Read the model definition and answer for the solid it produces. Units are mm, in the model's axes. A direction names the side the tool comes from. Coordinates: 2 decimals unless noted, no trailing zeros. Write each loop counter-clockwise with the first axis right and the second up, starting at its lowest first coordinate (ties: lowest second). Pieces come first, ordered by that corner, then holes.
1) The part is cut by section C-C (x = -21). Determine the outline of the cut face in (y, z), then the cut area to 3 significant figures.
2) Determine the mould class of faces 6 (the face through (-20.6, 18.5, 3.5)), 7 (the face through (-16, 10, 10)), 8 (the face through (-25, 10, 5)) for opening direction X: +X half, -X half, draft (parallel to the pull), parting line (faces both ways), or undercut.
3) The part is cut by section A-A (y = 16). Determine the outline of the cut face in (x, z).
4) The part is cut by section B-B (z = 6). Determine the outline of the cut face in (x, y).
5) Each of these flat-tipped pins is pushed along its axis until it touches: pin 1 Ø2.5 at (x, y) = (19.5, 16.5) entering from -Z; pin 2 Ø5.5 at (x, z) = (21, 8) entering from +Y; pin 3 Ø1.5 at (x, y) = (-4, 13.5) entering from +Z; pin 4 Ø2.5 at (x, y) = (-19.5, 7.5) entering from -Z. Where does it stop, or does it pass through?
6) Which of the six approach directions +Z, -Z, +X, -X, +Y, -Y give full straight-line access (tool end or side, diameter ignored) to faces 1 (the face through (20, 17, 3)), 2 (the face through (21, 15, 5)), 3 (the face through (-22.19, 12.88, 13.33)), 4 (the face through (16.305, 5.968, -6.563)), 5 (the face through (16, 9, 10))?
7) The part is cut by section D-D (y = 1.75). Determine the outline of the cut face in (x, z).
8) Find the intervals of material crossed by line 1 (Y direction, x = 20, z = -7); line 2 (Y direction, x = -21, z = 13.2); line 3 (X direction, y = 8.25, z = -1), in increasing order.
from build123d import *

# Parameters (mm, degrees)
BOSS_EXTRUDE1_DEPTH   = 15
CHAMFER1_SIZE         = 10
CHAMFER1_SIZE2        = 15
CHAMFER2_SIZE         = 15
CHAMFER2_SIZE2        = 10
SKETCH2_R             = 2.25
CUT_EXTRUDE1_DEPTH    = 36
SKETCH3_R             = 4
CUT_EXTRUDE2_DEPTH    = 13
SKETCH12_R            = 3
CUT_EXTRUDE7_DEPTH    = 4.2
M3_TAPPED_HOLE1_D     = 2.5
M3_TAPPED_HOLE1_DEPTH = 7.5
M3_TAPPED_HOLE1_TIP   = 0.751075774
M3_TAPPED_HOLE2_D     = 2.5
M3_TAPPED_HOLE2_DEPTH = 7.5
M3_TAPPED_HOLE2_TIP   = 0.751075774
BOSS_EXTRUDE3_START   = 4
SKETCH17_W            = 9
SKETCH17_H            = 13
SKETCH17_R            = 3
BOSS_EXTRUDE3_DEPTH   = 4
SKETCH18_R            = 5
CUT_EXTRUDE8_DEPTH    = 8.2
CHAMFER3_SIZE         = 1


with BuildPart() as part:
    # Sketch1 → Boss-Extrude1 (new body)
    with BuildSketch(Plane(origin=(0, 0, 0), x_dir=(1, 0, 0), z_dir=(0, 1, 0))):
        Polygon((-25, 16), (25, 16), (25, -16), (16, -16), (16, -3), (-16, -3), (-16, -16), (-25, -16), align=None)
    extrude(amount=BOSS_EXTRUDE1_DEPTH)

    # Chamfer1
    chamfer1_edges = [part.edges().sort_by_distance(p)[0] for p in [
        (25, 7.5, -16),
    ]]
    chamfer1_side = [part.faces().sort_by_distance(p)[0] for p in [
        (25, 7.5, 0),
    ]]
    chamfer(chamfer1_edges, length=CHAMFER1_SIZE, length2=CHAMFER1_SIZE2, reference=chamfer1_side[0])

    # Chamfer2
    chamfer2_edges = [part.edges().sort_by_distance(p)[0] for p in [
        (-25, 7.5, -16),
    ]]
    chamfer2_side = [part.faces().sort_by_distance(p)[0] for p in [
        (-7.5, 7.5, -16),
    ]]
    chamfer(chamfer2_edges, length=CHAMFER2_SIZE, length2=CHAMFER2_SIZE2, reference=chamfer2_side[0])

    # Sketch2 → Cut-Extrude1 (cut)
    with BuildSketch(Plane(origin=(0, 0, -16), x_dir=(-1, 0, 0), z_dir=(0, 0, -1))):
        with Locations((-20, 7.5)):
            Circle(SKETCH2_R)
        with Locations((20, 7.5)):
            Circle(SKETCH2_R)
    extrude(amount=-CUT_EXTRUDE1_DEPTH, mode=Mode.SUBTRACT)

    # Sketch3 → Cut-Extrude2 (cut)
    with BuildSketch(Plane(origin=(0, 0, -16), x_dir=(-1, 0, 0), z_dir=(0, 0, -1))):
        with Locations((-20, 7.5)):
            Circle(SKETCH3_R)
        with Locations((20, 7.5)):
            Circle(SKETCH3_R)
    extrude(amount=-CUT_EXTRUDE2_DEPTH, mode=Mode.SUBTRACT)

    # Sketch12 → Cut-Extrude7 (cut)
    with BuildSketch(Plane(origin=(0, 15, 0), x_dir=(1, 0, 0), z_dir=(0, 1, 0))):
        with Locations(Location((-21, -8, 0), (0, 0, 270))):
            Circle(SKETCH12_R)
        with Locations(Location((21, -8, 0), (0, 0, 270))):
            Circle(SKETCH12_R)
    extrude(amount=-CUT_EXTRUDE7_DEPTH, mode=Mode.SUBTRACT)

    # M3 Tapped Hole1
    with Locations(Plane(origin=(-21, 12.5, 16), x_dir=(1, 0, 0), z_dir=(0, 0, 1))):
        with Locations((0, 0)):
            Hole(M3_TAPPED_HOLE1_D / 2, depth=M3_TAPPED_HOLE1_DEPTH)
            with Locations((0, 0, -(M3_TAPPED_HOLE1_DEPTH + M3_TAPPED_HOLE1_TIP / 2))):  # 118° drill point
                Cone(0, M3_TAPPED_HOLE1_D / 2, M3_TAPPED_HOLE1_TIP, mode=Mode.SUBTRACT)

    # M3 Tapped Hole2
    with Locations(Plane(origin=(21, 12.5, 16), x_dir=(1, 0, 0), z_dir=(0, 0, 1))):
        with Locations((0, 0)):
            Hole(M3_TAPPED_HOLE2_D / 2, depth=M3_TAPPED_HOLE2_DEPTH)
            with Locations((0, 0, -(M3_TAPPED_HOLE2_DEPTH + M3_TAPPED_HOLE2_TIP / 2))):  # 118° drill point
                Cone(0, M3_TAPPED_HOLE2_D / 2, M3_TAPPED_HOLE2_TIP, mode=Mode.SUBTRACT)

    # Sketch17 → Boss-Extrude3 (add)
    # profile 1 of 2: a face of its own
    with BuildSketch(Plane(origin=(0, 15, 0), x_dir=(1, 0, 0), z_dir=(0, 1, 0)).offset(BOSS_EXTRUDE3_START)):
        with Locations((-20.5, -9.5)):
            Rectangle(SKETCH17_W, SKETCH17_H)
        with Locations(Location((-21, -8, 0), (0, 0, 270))):
            Circle(SKETCH17_R, mode=Mode.SUBTRACT)
    # profile 2 of 2: a face of its own
    with BuildSketch(Plane(origin=(0, 15, 0), x_dir=(1, 0, 0), z_dir=(0, 1, 0)).offset(BOSS_EXTRUDE3_START)):
        with Locations((20.5, -9.5)):
            Rectangle(SKETCH17_W, SKETCH17_H)
        with Locations(Location((21, -8, 0), (0, 0, 270))):
            Circle(SKETCH17_R, mode=Mode.SUBTRACT)
    extrude(amount=-BOSS_EXTRUDE3_DEPTH)

    # Sketch18 → Cut-Extrude8 (cut)
    with BuildSketch(Plane.XZ):
        with Locations(Location((0, -7.5, 0), (0, 0, 270))):
            Circle(SKETCH18_R)
    extrude(amount=-CUT_EXTRUDE8_DEPTH, mode=Mode.SUBTRACT)

    # Chamfer3
    chamfer3_edges = [part.edges().sort_by_distance(p)[0] for p in [
        (-20.5, 19, 3),
        (20.5, 19, 3),
        (-20.5, 19, 16),
        (20.5, 19, 16),
        (-25, 0, 5),
        (25, 0, 5),
    ]]
    chamfer(chamfer3_edges, length=CHAMFER3_SIZE)


solid = part.part
Reported:
1. outline: (0, -8.67) - (3.63, -8.67) - (3.63, -3) - (5.48, -3) - (5.48, 16) - (0, 16) - close; (9.52, -3) - (11.37, -3) - (11.37, -8.67) - (15, -8.67) - (15, 3) - (18, 3) - (19, 4) - (19, 5) - (10.8, 5) - (10.8, 11) - (11.25, 11) - (11.25, 16) - (9.52, 16) - close; (13.75, 11) - (19, 11) - (19, 15) - (18, 16) - (13.75, 16) - close
1. area: 239 mm2
2. face 6: draft
2. face 7: undercut
2. face 8: -X half
3. outline: (-25, 3) - (-16, 3) - (-16, 16) - (-25, 16) - close; (16, 3) - (25, 3) - (25, 16) - (16, 16) - close; hole circle Ø6 at (-21, 8); hole circle Ø6 at (21, 8)
4. outline: (-25, 1) - (-24, 0) - (-16, 0) - (-16, 19) - (-18.76, 19) - (-18.76, 10.8) - (-23.24, 10.8) - (-23.24, 19) - (-25, 19) - close; (16, 0) - (24, 0) - (25, 1) - (25, 19) - (23.24, 19) - (23.24, 10.8) - (18.76, 10.8) - (18.76, 19) - (16, 19) - close; hole circle Ø4.5 at (-20, 7.5); hole circle Ø4.5 at (20, 7.5)
5. pin 1: stops at z = 3
5. pin 2: stops at y = 10.8
5. pin 3: stops at z = 3
5. pin 4: passes through
6. face 1: -Z, +X, -X, +Y
6. face 2: +Y
6. face 3: +Z
6. face 4: -Z
6. face 5: +Z, +Y, -Y
7. outline: (-25, -6) - (-10, -16) - (10, -16) - (25, -6) - (25, 16) - (16, 16) - (16, 3) - (-16, 3) - (-16, 16) - (-25, 16) - close; hole circle Ø10 at (0, -7.5)
8. line 1: y = 0 to 3.5, 11.5 to 15
8. line 2: y = 0 to 5.48, 9.52 to 11.25, 13.75 to 19
8. line 3: x = -25 to -22.12, -17.88 to 17.88, 22.12 to 25
